For this review, take the finished solid that the model builds, in its own axes (mm). A direction names the side the tool comes from. Coordinates: 2 decimals unless noted, no trailing zeros. Write each loop counter-clockwise with the first axis right and the second up, starting at its lowest first coordinate (ties: lowest second). Pieces come first, ordered by that corner, then holes. Notation, with made-up numbers: M -17.75,1.5 L 26.25,1.5 A18 ccw 26.25,13.5 Z; hole C 44.5,65.25 d8. An arc over 180 degrees is marked long. Return JSON: item names as keys, results as strings.
```python
from build123d import *

# Parameters (mm, degrees)
SKETCH1_W           = 500
SKETCH1_H           = 320
SKETCH1_W_2         = 484
SKETCH1_H_2         = 304
BOSS_EXTRUDE1_DEPTH = 252.7


with BuildPart() as part:
    # Sketch1 → Boss-Extrude1 (new body)
    with BuildSketch(Plane.XY):
        with Locations((250, 160)):
            Rectangle(SKETCH1_W, SKETCH1_H)
        with Locations((250, 160)):
            Rectangle(SKETCH1_W_2, SKETCH1_H_2, mode=Mode.SUBTRACT)
    extrude(amount=BOSS_EXTRUDE1_DEPTH)


solid = part.part
```
1. We need section C-C (z = 36). State the section outline as (x, y) points, plus the area to 3 significant figures.
Checks:
{"outline": "M 0,0 L 500,0 L 500,320 L 0,320 Z; hole M 8,8 L 492,8 L 492,312 L 8,312 Z", "area": "12,900 mm2"}
2. For faces 1 (the face through (247, 0, 125)), 2 (the face through (247, 8, 125)), list the 3-axis set-ups (+Z, -Z, +X, -X, +Y, -Y) from which the entire face can be reached by the end or side of a thin tool; tool diameter is ignored.
Checks:
{"face 1": "+Z, -Z, +X, -X, -Y", "face 2": "+Z, -Z"}
3. We need section A-A (y = 291). State the section outline as (x, z) points.
Checks:
{"outline": "M 0,0 L 8,0 L 8,252.7 L 0,252.7 Z; M 492,0 L 500,0 L 500,252.7 L 492,252.7 Z"}
4. Wall thickness on L1, parallel to Y at x = 299.5, z = 95; L2, parallel to X at y = 140, z = 167: over which ranges is each line inside the solid? List them lowest first. Write a range as from..to.
Checks:
{"L1": "0..8, 312..320", "L2": "0..8, 492..500"}
5. We need section B-B (x = 322.5). State the section outline as (y, z) points.
Checks:
{"outline": "M 0,0 L 8,0 L 8,252.7 L 0,252.7 Z; M 312,0 L 320,0 L 320,252.7 L 312,252.7 Z"}
6. Draft analysis for pull direction X (two halves, no side actions). For faces 3 (the face through (492, 158, 125)), 4 (the face through (0, 158, 125)), 5 (the face through (247, 320, 125)), state which applies: +X half, -X half, draft (parallel to the pull), parting line (faces both ways), or undercut.
Checks:
{"face 3": "undercut", "face 4": "-X half", "face 5": "draft"}
